from build123d import *

# Parameters (mm, degrees)
SKETCH2_OUTSIDE_W              = 75.238
SKETCH2_OUTSIDE_H              = 75.238
SKETCH2_OUTSIDE_W_2            = 34
SKETCH2_OUTSIDE_H_2            = 60
CUT_EXTRUDE1_DEPTH             = 10
F_6_5_6_5_DIAMETER_HOLE1_D     = 6.5
F_6_5_6_5_DIAMETER_HOLE1_DEPTH = 20
F_6_5_6_5_DIAMETER_HOLE1_TIP   = 1.952797012
M20X1_5_TAPPED_HOLE1_D         = 18.5
M20X1_5_TAPPED_HOLE1_DEPTH     = 44.5
M20X1_5_TAPPED_HOLE1_TIP       = 5.557960726


with BuildPart() as part:
    # Sketch1 → Revolve1 (revolve)
    with BuildSketch(Plane.XY, mode=Mode.PRIVATE) as revolve1_sk:
        Polygon((0, 0), (28, 0), (28, 6), (14, 6), (14, 34), (0, 34), align=None)
    revolve(revolve1_sk.sketch.rotate(Axis((0, 34, 0), (0, -1, 0)), 180), axis=Axis((0, 34, 0), (0, -1, 0)))

    # Sketch2 outside → Cut-Extrude1 (cut)
    with BuildSketch(Plane.XZ):
        Rectangle(SKETCH2_OUTSIDE_W, SKETCH2_OUTSIDE_H)
        Rectangle(SKETCH2_OUTSIDE_W_2, SKETCH2_OUTSIDE_H_2, mode=Mode.SUBTRACT)
    extrude(amount=-CUT_EXTRUDE1_DEPTH, mode=Mode.SUBTRACT)

    # Ø6.5 (6.5) Diameter Hole1
    with Locations(Plane.XZ):
        with Locations((-10.5, 18.186533479), (10.5, 18.186533479), (-10.5, -18.186533479), (10.5, -18.186533479)):
            Hole(F_6_5_6_5_DIAMETER_HOLE1_D / 2, depth=F_6_5_6_5_DIAMETER_HOLE1_DEPTH)
            with Locations((0, 0, -(F_6_5_6_5_DIAMETER_HOLE1_DEPTH + F_6_5_6_5_DIAMETER_HOLE1_TIP / 2))):  # 118° drill point
                Cone(0, F_6_5_6_5_DIAMETER_HOLE1_D / 2, F_6_5_6_5_DIAMETER_HOLE1_TIP, mode=Mode.SUBTRACT)

    # M20x1.5 Tapped Hole1
    with Locations(Plane.XZ):
        with Locations((0, 0)):
            Hole(M20X1_5_TAPPED_HOLE1_D / 2, depth=M20X1_5_TAPPED_HOLE1_DEPTH)
            with Locations((0, 0, -(M20X1_5_TAPPED_HOLE1_DEPTH + M20X1_5_TAPPED_HOLE1_TIP / 2))):  # 118° drill point
                Cone(0, M20X1_5_TAPPED_HOLE1_D / 2, M20X1_5_TAPPED_HOLE1_TIP, mode=Mode.SUBTRACT)


solid = part.part
Check sheet for the modelled part. Datum: model origin and axes. Units: mm. A direction names the side the tool comes from. Round coordinates to 2 decimals unless told otherwise and drop trailing zeros. Order: outer loops, then holes, each group sorted by start corner. A loop starts at its lowest first (then second) coordinate and runs counter-clockwise, first axis right, second up. Notation, with made-up numbers: M 21,-5 L 31,-5 A19 cw 31,27 Z; hole C 25.5,-38.75 d5. An arc over 180 degrees is marked long. One line per item, written item: value. Start each with the question number.
1. Section check D-D on y = 3.5. Enter the section's corners in (x, z), and give its area (3 significant figures).
2. Release check for a two-part mould opening along Z. For faces 1 (the cylindrical face through (2.01, 17.24, -9.03)), 2 (the flat face through (-17, 3, 0)), 3 (the cylindrical face through (0, 3, -28)) record: released by +Z, released by -Z, zero draft, split by the parting line, or undercut.
3. Access from +Z, -Z, +X, -X, +Y, -Y to the whole of each face (thin tool, end or side, straight path). Record for faces 4 (the flat face through (17, 3, 0)), 5 (the flat face through (-7, 6, -13)).
4. Section check A-A on z = 0. Enter the section's corners in (x, y).
5. Section check B-B on x = 0. Enter the section's corners in (y, z).
6. Scan lines: line 1 along Z through (x, y) = (10.5, 1.55); line 2 along X through (y, z) = (16, 0.5); line 3 along Z through (x, y) = (5.5, 21.5). Record each from-to range of solid material in increasing order.
7. Section check C-C on x = -10.5. Enter the section's corners in (y, z).
8. Gauge pin test, flat ends, axial feed: P1, Ø8, axis at x = -11, y = 20.5, coming from the -Z side; P2, Ø11, axis at x = 0, z = 0, coming from the -Y side; P3, Ø4, axis at y = 8.5, z = 12.5, coming from the +X side; P4, Ø12, axis at x = -9.5, y = 18.5, coming from the +Z side. Record the tip position at first contact, or that the pin passes through.
Results found:
1. outline: M -17,-22.25 A28 ccw 17,-22.25 L 17,22.25 A28 ccw -17,22.25 Z; hole C -10.5,-18.19 d6.5; hole C -10.5,18.19 d6.5; hole C 0,0 d18.5; hole C 10.5,-18.19 d6.5; hole C 10.5,18.19 d6.5
1. area: 1,380 mm^2
2. face 1: undercut
2. face 2: zero draft
2. face 3: released by -Z
3. face 4: +Z, -Z, +X, +Y, -Y
3. face 5: +Y
4. outline: M -17,0 L -9.25,0 L -9.25,34 L -14,34 L -14,6 L -17,6 Z; M 9.25,0 L 17,0 L 17,6 L 14,6 L 14,34 L 9.25,34 Z
5. outline: M 0,-28 L 6,-28 L 6,-14 L 34,-14 L 34,-9.25 L 0,-9.25 Z; M 0,9.25 L 34,9.25 L 34,14 L 6,14 L 6,28 L 0,28 Z
6. line 1: -25.96 to -21.44, -14.94 to 14.94, 21.44 to 25.96
6. line 2: -13.99 to -9.24, 9.24 to 13.99
6. line 3: -12.87 to -7.44, 7.44 to 12.87
7. outline: M 0,-25.96 L 6,-25.96 L 6,-21.44 L 0,-21.44 Z; M 0,-14.94 L 6,-14.94 L 6,-9.26 L 34,-9.26 L 34,9.26 L 6,9.26 L 6,14.94 L 0,14.94 Z; M 0,21.44 L 6,21.44 L 6,25.96 L 0,25.96 Z
8. P1: z = -12.12
8. P2: through
8. P3: x = 9.26
8. P4: z = 13.56
